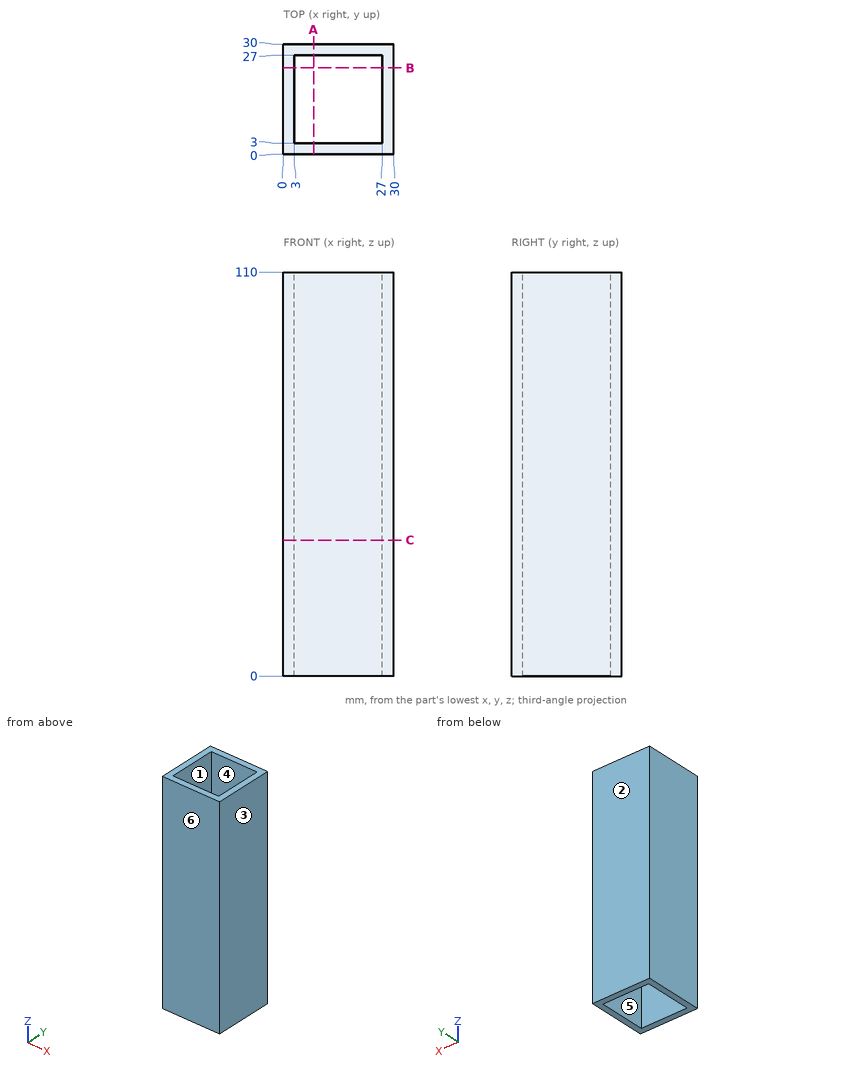
Verification items for this drawing (mm, ordinates from the low corner). A direction names the side the tool comes from. Round coordinates to 2 decimals unless told otherwise and drop trailing zeros. Loops run counter-clockwise (first coordinate to the right, second up) from the corner with the lowest first, then second, coordinate; pieces in that order, holes last. Notation, with made-up numbers: M 65.5,39 L 106.5,39 A26 ccw 106.5,69 Z; hole C 60,-10 d9. An arc over 180 degrees is marked long. Answer as a JSON object with one key per item and string values.
1. Mould release check, pull along X, two halves, no side actions. Record for the marked faces 1, 2, 3 and 4: pulls with the +X half, pulls with the -X half, needs draft (parallel to the pull), parting line crosses it, or undercut.
Reply:
{"face 1": "undercut", "face 2": "needs draft", "face 3": "pulls with the +X half", "face 4": "undercut"}
2. Scan line: line 1 (Y direction, x = 23.5, z = 23). Record every from-to range of solid material in increasing order.
Reply:
{"line 1": "y = 0 to 3, 27 to 30"}
3. Section check A-A (x = 8.25). Record the boundary of the cut face in (y, z), plus the area to 3 significant figures.
Reply:
{"outline": "M 0,0 L 3,0 L 3,110 L 0,110 Z; M 27,0 L 30,0 L 30,110 L 27,110 Z", "area": "660 mm²"}
4. Gauge pin test, flat end, axial feed: P1, Ø12, axis at x = 18.5, y = 19, coming from the -Z side. Record the tip position at first contact, or that the pin passes through.
Reply:
{"P1": "passes through"}
5. Section check C-C (z = 37). Record the boundary of the cut face in (x, y).
Reply:
{"outline": "M 0,0 L 30,0 L 30,30 L 0,30 Z; hole M 3,3 L 27,3 L 27,27 L 3,27 Z"}
6. Access from +Z, -Z, +X, -X, +Y, -Y to the whole of each face (thin tool, end or side, straight path). Record for the marked faces 5 and 6.
Reply:
{"face 5": "+Z, -Z", "face 6": "+Z, -Z, +X, -X, -Y"}
